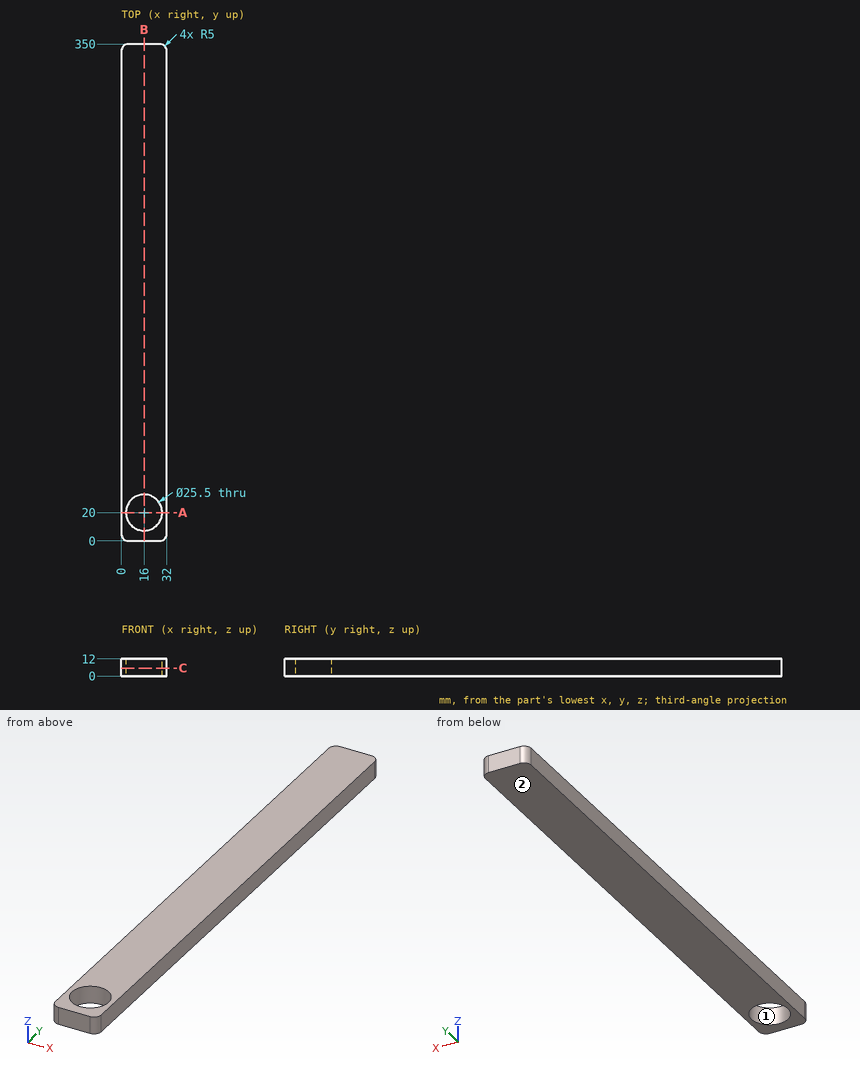
Print and shaded views of the part. All mm, measured from the part's lowest x, y and z. Coordinates: 2 decimals unless noted, no trailing zeros. Order: outer loops, then holes, each group sorted by start corner. A loop starts at its lowest first (then second) coordinate and runs counter-clockwise, first axis right, second up. Notation, with made-up numbers: (43.25, -17) -> (74.25, -17) arc R27 cw to (74.25, 12) -> close; hole circle Ø10 at (18, 47.5). An arc over 180 degrees is marked (long way). Answer as a JSON object with one key per item and string values. Group by question number.
1) Drill centre lines: L1, parallel to Y at x = 16, z = 5.25; L2, parallel to Y at x = 9, z = 10.75; L3, parallel to Y at x = 3, z = 5.75. Where is each one in solid material? Low to high.
2) Cut at B-B, the plane x = 16. Write the cut outline in (y, z).
3) Pull direction X, two halves, no side cores. Call the marked faces 1 and 2: +X half, -X half, draft (parallel to the pull), parting line (faces both ways), or undercut.
4) Cut at C-C, the plane z = 5.5. Write the cut outline in (x, y).
5) Cut at A-A, the plane y = 20. Write the cut outline in (x, z).
Check values:
{
 "1": {"L1": "y = 0 to 7.25, 32.75 to 350", "L2": "y = 0 to 9.34, 30.66 to 350", "L3": "y = 0.42 to 349.58"},
 "2": {"outline": "(0, 0) -> (7.25, 0) -> (7.25, 12) -> (0, 12) -> close; (32.75, 0) -> (350, 0) -> (350, 12) -> (32.75, 12) -> close"},
 "3": {"face 1": "undercut", "face 2": "draft"},
 "4": {"outline": "(0, 5) arc R5 ccw to (5, 0) -> (27, 0) arc R5 ccw to (32, 5) -> (32, 345) arc R5 ccw to (27, 350) -> (5, 350) arc R5 ccw to (0, 345) -> close; hole circle Ø25.5 at (16, 20)"},
 "5": {"outline": "(0, 0) -> (3.25, 0) -> (3.25, 12) -> (0, 12) -> close; (28.75, 0) -> (32, 0) -> (32, 12) -> (28.75, 12) -> close"}
}
